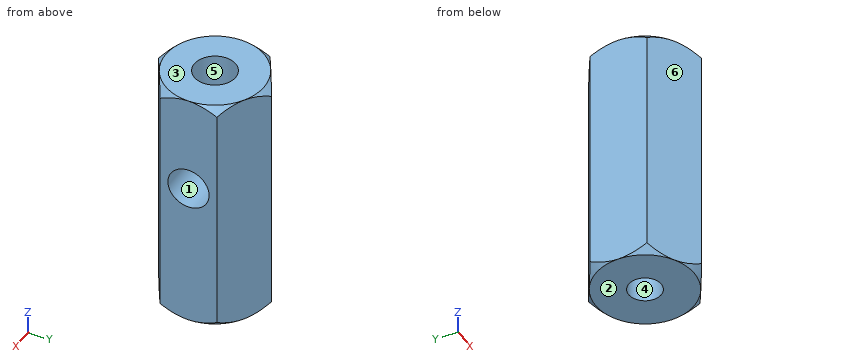
```python
from build123d import *

# Parameters (mm, degrees)
BOSS_EXTRUDE1_DEPTH   = 25
M5_TAPPED_HOLE3_D     = 4.2
M5_TAPPED_HOLE3_DEPTH = 10
M5_TAPPED_HOLE3_TIP   = 1.2618073
M4_TAPPED_HOLE1_D     = 3.3
M4_TAPPED_HOLE1_DEPTH = 9
M4_TAPPED_HOLE1_TIP   = 0.991420021
SKETCH7_W             = 2.1
SKETCH7_H             = 5


with BuildPart() as part:
    # Sketch1 → Boss-Extrude1 (new body)
    with BuildSketch(Plane.XY):
        Polygon((0, 5.773502692), (-5, 2.886751346), (-5, -2.886751346), (0, -5.773502692), (5, -2.886751346), (5, 2.886751346), align=None)
    extrude(amount=BOSS_EXTRUDE1_DEPTH)

    # M5 Tapped Hole3
    with Locations(Plane.XY.offset(25)):
        with Locations((0, 0)):
            Hole(M5_TAPPED_HOLE3_D / 2, depth=M5_TAPPED_HOLE3_DEPTH)
            with Locations((0, 0, -(M5_TAPPED_HOLE3_DEPTH + M5_TAPPED_HOLE3_TIP / 2))):  # 118° drill point
                Cone(0, M5_TAPPED_HOLE3_D / 2, M5_TAPPED_HOLE3_TIP, mode=Mode.SUBTRACT)

    # M4 Tapped Hole1
    with Locations(Plane(origin=(0, 0, 0), x_dir=(-1, 0, 0), z_dir=(0, 0, -1))):
        with Locations((0, 0)):
            Hole(M4_TAPPED_HOLE1_D / 2, depth=M4_TAPPED_HOLE1_DEPTH)
            with Locations((0, 0, -(M4_TAPPED_HOLE1_DEPTH + M4_TAPPED_HOLE1_TIP / 2))):  # 118° drill point
                Cone(0, M4_TAPPED_HOLE1_D / 2, M4_TAPPED_HOLE1_TIP, mode=Mode.SUBTRACT)

    # Sketch7 → M5 Tapped Hole2 (revolve, cut)
    with BuildSketch(Plane(origin=(0, 0, 15), x_dir=(0, 0, 1), z_dir=(0, 1, 0))):
        with Locations((1.05, 2.5)):
            Rectangle(SKETCH7_W, SKETCH7_H)
    revolve(axis=Axis((-6.35, 0, 15), (1, 0, 0)), mode=Mode.SUBTRACT)

    # Sketch8 → Cut-Revolve1 (revolve, cut)
    with BuildSketch(Plane(origin=(0, 0, 0), x_dir=(0, 0, -1), z_dir=(1, 0, 0)), mode=Mode.PRIVATE) as cut_revolve1_sk:
        Polygon((-25, 5), (-25, 5.773502692), (-24.226497308, 5.773502692), align=None)
        Polygon((0, 5), (0, 5.773502692), (-0.773502692, 5.773502692), align=None)
    revolve(cut_revolve1_sk.sketch.rotate(Axis((0, 0, 25), (0, 0, -1)), 90), axis=Axis((0, 0, 25), (0, 0, -1)), mode=Mode.SUBTRACT)


solid = part.part
```
Can you work these out from the model? Positions are in its coordinate system, mm. Face numbers are marked on the shaded views. A direction names the side the tool comes from. Give positions to 0.01 mm unless a question says otherwise; leave off trailing zeros. Loops run counter-clockwise (first coordinate to the right, second up) from the corner with the lowest first, then second, coordinate; pieces in that order, holes last. Notation, with made-up numbers: M -16,65.5 L 5,65.5 A33 cw 5,100.5 Z; hole C 0,81 d10. An arc over 180 degrees is marked long. Use CSV: the item, a comma, the result in double quotes. Start each with the question number.
1. On a 3-axis mill with a long thin cutter (end or side, diameter ignored), from which of +Z, -Z, +X, -X, +Y, -Y can I reach the whole of each face in a straight line? I mean the marked faces 5 and 6. Say none if no direction works.
2. If I drill on L1, parallel to X at y = 0, z = 20.75; L2, parallel to Z at x = 2.5, y = -0.75; L3, parallel to X at y = -0.75, z = 5, over which ranges is the centre line in solid material (lowest first)?
3. Imagine slicing it at A-A, the plane z = 5.25. Write out the boundary of the cut face in (x, y), plus the area to 3 significant figures.
4. If we mould it in two halves opening along Z, with no side actions, what happens to the marked faces 1, 2, 3 and 4? For each: released by +Z, released by -Z, zero draft, split by the parting line, or undercut.
5. Imagine slicing it at B-B, the plane z = 20. Write out the boundary of the cut face in (x, y).
6. For P1, Ø5, axis at x = 1, z = 5.5, coming from the +Y side; P2, Ø2, axis at x = 0, y = 0, coming from the +Z side; P3, Ø5, axis at x = 3.5, z = 12.5, coming from the -Y side; P4, Ø5, axis at x = 0, y = 0, coming from the -Z side, each with a flat end and sliding along its axis, tell me the tip position at first contact or that it passes through.
Response values:
1,face 5,"+Z"
1,face 6,"+Z, -Z, -X, -Y"
2,L1,"-5 to -2.1, 2.1 to 5"
2,L2,"0 to 13.04, 16.96 to 25"
2,L3,"-5 to -1.47, 1.47 to 5"
3,outline,"M -5,-2.89 L 0,-5.77 L 5,-2.89 L 5,2.89 L 0,5.77 L -5,2.89 Z; hole C 0,0 d3.3"
3,area,"78.0 mm^2"
4,face 1,"undercut"
4,face 2,"released by -Z"
4,face 3,"released by +Z"
4,face 4,"zero draft"
5,outline,"M -5,-2.89 L 0,-5.77 L 5,-2.89 L 5,2.89 L 0,5.77 L -5,2.89 Z; hole C 0,0 d4.2"
6,P1,"y = 5.77"
6,P2,"z = 14.34"
6,P3,"y = -5.2"
6,P4,"z = 0"
